Model file for the job. Use its own axes, mm. Face numbers are marked on the shaded views. A direction names the side the tool comes from. Coordinates: 2 decimals unless noted, no trailing zeros. Write each loop counter-clockwise with the first axis right and the second up, starting at its lowest first coordinate (ties: lowest second). Pieces come first, ordered by that corner, then holes.
Q1. Band-saw the part on B-B, the plane x = 8.5. Write the cut outline in (y, z).
Q2. Drill centre lines: probe 1 along Z at (x, y) = (0, -46); probe 2 along Y at (x, z) = (-71.75, 10); probe 3 along Y at (x, z) = (0.5, 2.75). Where is each one in solid material? Low to high.
Q3. Band-saw the part on A-A, the plane y = 11. Write the cut outline in (x, z).
Q4. Pin check, flat tips, straight feed: P1, Ø5.5, axis at x = 0, z = 10.5, coming from the +Y side; P2, Ø10, axis at x = 0.5, y = -38.5, coming from the -Z side; P3, Ø3, axis at x = -66.5, z = 10.5, coming from the +Y side. Stop position of each tip, or through.
Q5. Which spindle directions (+Z, -Z, +X, -X, +Y, -Y) get a long thin tool onto all of the face, cutting with end or side? Do the marked faces 1 and 2. Say none if no direction does.
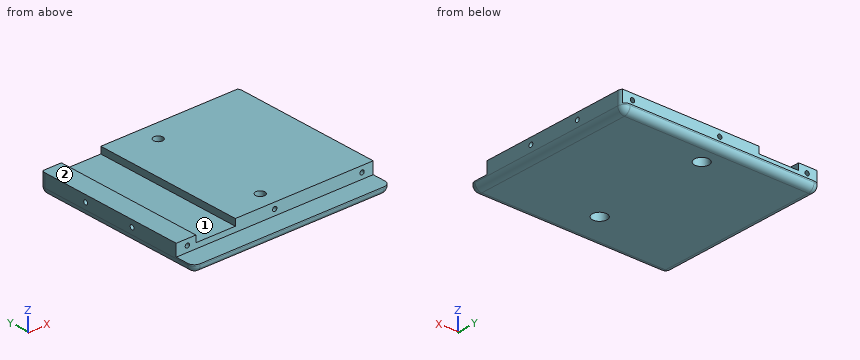
from build123d import *

# Parameters (mm, degrees)
SKETCH_1_W                  = 150
SKETCH_1_H                  = 133
EXTRUDE_1_DEPTH             = 15
SKETCH_2_W                  = 23.680798508
SKETCH_2_H                  = 30.226028772
CUT_EXTRUDE_1_DEPTH         = 165.764225486
FILLET_2_R                  = 5
HOLE_WIZARD_2_D             = 7
HOLE_WIZARD_2_CBORE_D       = 11
HOLE_WIZARD_2_CBORE_DEPTH   = 7
SKETCH_19_W                 = 244.102436516
SKETCH_19_H                 = 114.665953459
CUT_EXTRUDE_7_DEPTH         = 15
SKETCH_29_W                 = 30
SKETCH_29_H                 = 229.451153657
CUT_EXTRUDE_11_DEPTH        = 5
HOLE_WIZARD_M4_1_D          = 3.3
HOLE_WIZARD_M4_1_DEPTH      = 12
HOLE_WIZARD_M4_1_TIP        = 0.991420021
HOLE_WIZARD_M4_2_D          = 3.3
HOLE_WIZARD_M4_2_DEPTH      = 12
HOLE_WIZARD_M4_2_TIP        = 0.991420021
HOLE_WIZARD_M4_3_AT_2_COUNT = 2
HOLE_WIZARD_M4_3_AT_2_PITCH = 40


with BuildPart() as part:
    # 草图1 → 凸台-拉伸1 (new body)
    with BuildSketch(Plane.XY):
        Rectangle(SKETCH_1_W, SKETCH_1_H)
    extrude(amount=EXTRUDE_1_DEPTH)

    # 草图2 → 切除-拉伸1 (cut, through all)
    with BuildSketch(Plane.ZY.offset(75)):
        with Locations((17.840399254, 79.613014386)):
            Rectangle(SKETCH_2_W, SKETCH_2_H)
    extrude(amount=-CUT_EXTRUDE_1_DEPTH, mode=Mode.SUBTRACT)

    # 圆角2
    fillet_2_edges = [part.edges().sort_by_distance(p)[0] for p in [
        (-75, 66.5, 3),
        (-75, 0, 0),
        (-75, -66.5, 7.5),
        (0, -66.5, 0),
        (75, -66.5, 7.5),
        (75, 0, 0),
        (75, 66.5, 3),
        (0, 66.5, 0),
    ]]
    fillet(fillet_2_edges, radius=FILLET_2_R)

    # 打孔尺寸(%根据)开槽圆柱头螺钉的类型2 (through all)
    with Locations(Plane(origin=(0, 0, 0), x_dir=(-1, 0, 0), z_dir=(0, 0, -1))):
        with Locations((-0.5, 49.5), (-0.5, -38.5)):
            CounterBoreHole(HOLE_WIZARD_2_D / 2, HOLE_WIZARD_2_CBORE_D / 2, HOLE_WIZARD_2_CBORE_DEPTH)

    # 草图19 → 切除-拉伸7 (cut)
    with BuildSketch(Plane.XZ.offset(66.5)):
        with Locations((-15.450751356, 63.33297673)):
            Rectangle(SKETCH_19_W, SKETCH_19_H)
    extrude(amount=-CUT_EXTRUDE_7_DEPTH, mode=Mode.SUBTRACT)

    # 草图29 → 切除-拉伸11 (cut)
    with BuildSketch(Plane.XY.offset(15)):
        with Locations((-45, 14.041040746)):
            Rectangle(SKETCH_29_W, SKETCH_29_H)
    extrude(amount=-CUT_EXTRUDE_11_DEPTH, mode=Mode.SUBTRACT)

    # M4 螺纹孔1
    with Locations(Plane(origin=(0, -51.5, 0), x_dir=(-1, 0, 0), z_dir=(0, -1, 0))):
        with Locations((66.5, -10.5), (-66.5, -10.5), (0, -10.5)):
            Hole(HOLE_WIZARD_M4_1_D / 2, depth=HOLE_WIZARD_M4_1_DEPTH)
            with Locations((0, 0, -(HOLE_WIZARD_M4_1_DEPTH + HOLE_WIZARD_M4_1_TIP / 2))):  # 118° drill point
                Cone(0, HOLE_WIZARD_M4_1_D / 2, HOLE_WIZARD_M4_1_TIP, mode=Mode.SUBTRACT)

    # M4 螺纹孔2
    with Locations(Plane(origin=(0, 64.5, 0), x_dir=(1, 0, 0), z_dir=(0, 1, 0))):
        with Locations((-66.5, -10.5), (66.5, -10.5), (0, -10.5)):
            Hole(HOLE_WIZARD_M4_2_D / 2, depth=HOLE_WIZARD_M4_2_DEPTH)
            with Locations((0, 0, -(HOLE_WIZARD_M4_2_DEPTH + HOLE_WIZARD_M4_2_TIP / 2))):  # 118° drill point
                Cone(0, HOLE_WIZARD_M4_2_D / 2, HOLE_WIZARD_M4_2_TIP, mode=Mode.SUBTRACT)

    # 草图37 → M4 螺纹孔3 (revolve, cut)
    with BuildSketch(Plane(origin=(-75, 26.61076125, 10), x_dir=(0, 0, 1), z_dir=(0, 1, 0))):
        Polygon((0, 0), (0, 12.991420021), (1.65, 12), (1.65, 0), align=None)
    hole_wizard_m4_3 = revolve(axis=Axis((-81.35, 26.61076125, 10), (1, 0, 0)), mode=Mode.SUBTRACT)

    # M4 螺纹孔3 at 2: M4 螺纹孔3 ×2
    with Locations(*[(0, -i * HOLE_WIZARD_M4_3_AT_2_PITCH, 0) for i in range(1, HOLE_WIZARD_M4_3_AT_2_COUNT)]):
        add(hole_wizard_m4_3, mode=Mode.SUBTRACT)

    # 镜向1: M4 螺纹孔3 across plane
    add(hole_wizard_m4_3.mirror(Plane(origin=(0, 0, 0), x_dir=(0, 0, 1), z_dir=(1, 0, 0))), mode=Mode.SUBTRACT)

    # 镜向1 copy 1 sketch → 镜向1 copy 1 (revolve, cut)
    with BuildSketch(Plane(origin=(75, -13.38923875, 10), x_dir=(0, 0, 1), z_dir=(0, 1, 0))):
        Polygon((0, 0), (0, -12.991420021), (1.65, -12), (1.65, 0), align=None)
    revolve(axis=Axis((81.35, -13.38923875, 10), (1, 0, 0)), mode=Mode.SUBTRACT)


solid = part.part
Answer sheet:
1. outline: (-66.5, 5) arc R5 ccw to (-61.5, 0) - (61.5, 0) arc R5 ccw to (66.5, 5) - (66.5, 6) - (64.5, 6) - (64.5, 15) - (-51.5, 15) - (-51.5, 6) - (-66.5, 6) - close
2. probe 1: z = 0 to 8.85, 12.15 to 15
2. probe 2: y = -51.5 to -15.04, -11.74 to 24.96, 28.26 to 64.5
2. probe 3: y = -65.97 to -44, -33 to 44, 55 to 65.97
3. outline: (-75, 5) arc R5 ccw to (-70, 0) - (70, 0) arc R5 ccw to (75, 5) - (75, 15) - (-30, 15) - (-30, 10) - (-60, 10) - (-60, 15) - (-75, 15) - close
4. P1: stops at y = 64.5
4. P2: stops at z = 7
4. P3: stops at y = 52.41
5. face 1: +Z, +Y, -Y
5. face 2: +Z, +X, -X, +Y, -Y
